Verification items for this drawing (mm, ordinates from the low corner). A direction names the side the tool comes from. Coordinates: 2 decimals unless noted, no trailing zeros. Write each loop counter-clockwise with the first axis right and the second up, starting at its lowest first coordinate (ties: lowest second). Pieces come first, ordered by that corner, then holes.
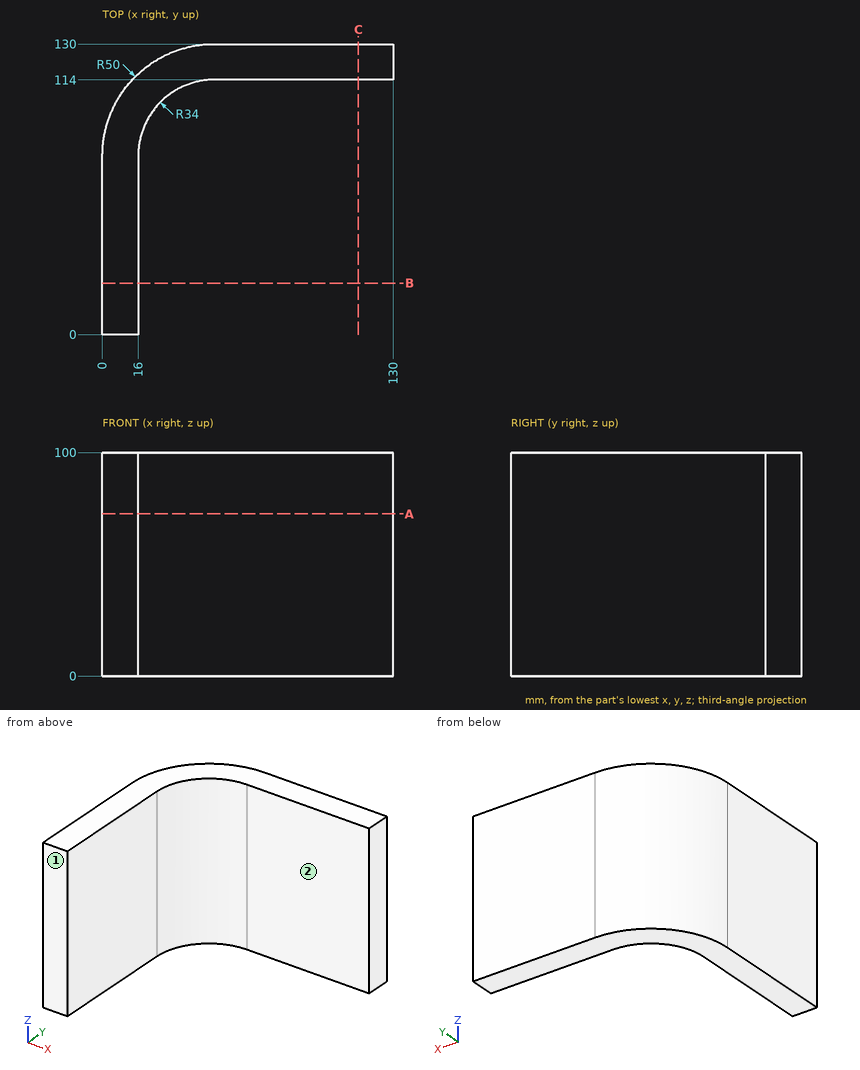
1. Sectioned sample at A-A, the plane z = 72.5. Record the boundary of the cut face in (x, y).
Computed values:
outline: (0, 0) - (16, 0) - (16, 80) arc R34 cw to (50, 114) - (130, 114) - (130, 130) - (50, 130) arc R50 ccw to (0, 80) - close
2. Access from +Z, -Z, +X, -X, +Y, -Y to the whole of each face (thin tool, end or side, straight path). Record for the marked faces 1 and 2.
Computed values:
face 1: +Z, -Z, +X, -X, -Y
face 2: +Z, -Z, +X, -Y
3. Sectioned sample at B-B, the plane y = 23. Record the boundary of the cut face in (x, z).
Computed values:
outline: (0, 0) - (16, 0) - (16, 100) - (0, 100) - close
4. Gauge pin test, flat ends, axial feed: pin 1 Ø10 at (y, z) = (75, 88.5) entering from +X; pin 2 Ø24 at (x, z) = (106.5, 27) entering from -Y; pin 3 Ø2 at (y, z) = (103, 49) entering from +X. Record the tip position at first contact, or that the pin passes through.
Computed values:
pin 1: stops at x = 16
pin 2: stops at y = 114
pin 3: stops at x = 25.92
5. Thickness scan on line 1 along Y through (x, z) = (118, 56.5); line 2 along X through (y, z) = (63, 64.5); line 3 along X through (y, z) = (120.5, 88). Record the ranges inside material, lowest first.
Computed values:
line 1: y = 114 to 130
line 2: x = 0 to 16
line 3: x = 20.68 to 130
6. Sectioned sample at C-C, the plane x = 114.5. Record the boundary of the cut face in (y, z).
Computed values:
outline: (114, 0) - (130, 0) - (130, 100) - (114, 100) - close
